from build123d import *

# Parameters (mm, degrees)
BASE_BLOCK_84MM_DEPTH  = 84
BACK_CHANNEL_SKETCH_W  = 12
BACK_CHANNEL_SKETCH_H  = 10
BACK_CHANNEL_CUT_DEPTH = 84
FRONT_PAD_SKETCH_W     = 8
FRONT_PAD_SKETCH_H     = 71
FRONT_PAD_8MM_DEPTH    = 15
TOP_CHAMFER_CUT_DEPTH  = 42.5
SLOT_CUT_DEPTH         = 75


with BuildPart() as part:
    # Block Profile Sketch → Base Block 84mm (new body)
    with BuildSketch(Plane.XY):
        Polygon((0, 0), (27, 0), (27, 71), (15, 71), (0, 60.496886927), (0, 52.496886927), (12, 52.496886927), (12, 15.496886927), (0, 15.496886927), align=None)
    extrude(amount=BASE_BLOCK_84MM_DEPTH)

    # Back Channel Sketch → Back Channel Cut (cut)
    with BuildSketch(Plane(origin=(0, 15.496886927, 0), x_dir=(1, 0, 0), z_dir=(0, 1, 0))):
        with Locations((6, -79)):
            Rectangle(BACK_CHANNEL_SKETCH_W, BACK_CHANNEL_SKETCH_H)
        with Locations((6, -5)):
            Rectangle(BACK_CHANNEL_SKETCH_W, BACK_CHANNEL_SKETCH_H)
    extrude(amount=BACK_CHANNEL_CUT_DEPTH, mode=Mode.SUBTRACT)

    # Front Pad Sketch → Front Pad 8mm (add, symmetric)
    with BuildSketch(Plane.XY.offset(42)):
        with Locations((31, 35.5)):
            Rectangle(FRONT_PAD_SKETCH_W, FRONT_PAD_SKETCH_H)
    extrude(amount=FRONT_PAD_8MM_DEPTH, both=True)

    # Top Chamfer Sketch → Top Chamfer Cut (cut, symmetric)
    with BuildSketch(Plane(origin=(27, 0, 0), x_dir=(0, 0, -1), z_dir=(1, 0, 0))):
        Polygon((-54.5, 71), (-74.175600087, 55.067013206), (-84, 39.938763989), (-84, 71), align=None)
        Polygon((-29.5, 71), (-9.824399913, 55.067013206), (0, 39.938763989), (0, 71), align=None)
    extrude(amount=TOP_CHAMFER_CUT_DEPTH, both=True, mode=Mode.SUBTRACT)

    # Slot Sketch → Slot Cut (cut)
    with BuildSketch(Plane.ZY.offset(-12)):
        with BuildLine():
            Line((46, 43.035553087), (46, 22.035553087))
            ThreePointArc((46, 22.035553087), (42, 18.035553087), (38, 22.035553087))
            Line((38, 22.035553087), (38, 43.035553087))
            ThreePointArc((38, 43.035553087), (42, 47.035553087), (46, 43.035553087))
        make_face()
    extrude(amount=-SLOT_CUT_DEPTH, mode=Mode.SUBTRACT)


solid = part.part
The listing builds one solid part. Answer for the finished solid, in the listing's coordinates (mm). A direction names the side the tool comes from. Round coordinates to 2 decimals unless told otherwise and drop trailing zeros. Loops run counter-clockwise (first coordinate to the right, second up) from the corner with the lowest first, then second, coordinate; pieces in that order, holes last. Notation, with made-up numbers: M 57.25,86 L 107.25,86 A17 cw 107.25,117 Z; hole C 38.5,63.5 d5. An arc over 180 degrees is marked long. Return JSON: item names as keys, results as strings.
Q1. Find section D-D, the plane x = 29.5. Determine the outline of the cut face in (y, z).
Results list:
{"outline": "M 0,27 L 68.98,27 L 71,29.5 L 71,54.5 L 68.98,57 L 0,57 Z; hole M 22.04,38 L 43.04,38 A4 ccw 43.04,46 L 22.04,46 A4 ccw Z"}
Q2. Which of the six approach directions +Z, -Z, +X, -X, +Y, -Y give full straight-line access (tool end or side, diameter ignored) to faces 4 (the face through (23.339, 18.037, 42.088)), 5 (the face through (27, 26, 13)), 6 (the face through (31, 35, 57))?
Results list:
{"face 4": "+X, -X", "face 5": "-Z, +X, +Y, -Y", "face 6": "+Z, +X, +Y, -Y"}
Q3. The mould has two halves that part along Z. Classify faces 1 (the face through (23.339, 47.035, 41.912)), 2 (the face through (35, 35, 49)), 3 (the face through (6, 54, 10)): released by +Z, released by -Z, zero draft, split by the parting line, or undercut.
Results list:
{"face 1": "undercut", "face 2": "zero draft", "face 3": "released by -Z"}
Q4. Find the intervals of material crossed by line 1 along Z through (x, y) = (22.5, 33.5); line 2 along Z through (x, y) = (28.5, 25); line 3 along X through (y, z) = (37.5, 59.5), in increasing order. Write a range as from..to.
Results list:
{"line 1": "z = 0..38, 46..84", "line 2": "z = 27..38, 46..57", "line 3": "x = 12..27"}
Q5. Find section A-A, the plane z = 42. Determine the outline of the cut face in (x, y).
Results list:
{"outline": "M 0,0 L 35,0 L 35,18.04 L 12,18.04 L 12,15.5 L 0,15.5 Z; M 0,52.5 L 12,52.5 L 12,47.04 L 35,47.04 L 35,71 L 15,71 L 0,60.5 Z"}
Q6. Find section C-C, the plane x = 17.5. Determine the outline of the cut face in (y, z), plus the area to 3 significant figures.
Results list:
{"outline": "M 0,0 L 39.94,0 L 55.07,9.82 L 71,29.5 L 71,54.5 L 55.07,74.18 L 39.94,84 L 0,84 Z; hole M 22.04,38 L 43.04,38 A4 ccw 43.04,46 L 22.04,46 A4 ccw Z", "area": "4,970 mm2"}
Q7. Each of these flat-tipped pins is pushed along its axis until it touches: pin 1 Ø5 at (x, y) = (13.5, 60.5) entering from +Z; pin 2 Ø3 at (x, y) = (5, 53) entering from -Z; pin 3 Ø6.5 at (x, y) = (30.5, 33) entering from +Z. Where does it stop, or does it pass through?
Results list:
{"pin 1": "stops at z = 70.55", "pin 2": "stops at z = 10", "pin 3": "stops at z = 57"}
Q8. Find section B-B, the plane y = 27.5. Determine the outline of the cut face in (x, z).
Results list:
{"outline": "M 12,0 L 27,0 L 27,27 L 35,27 L 35,38 L 12,38 Z; M 12,46 L 35,46 L 35,57 L 27,57 L 27,84 L 12,84 Z"}
